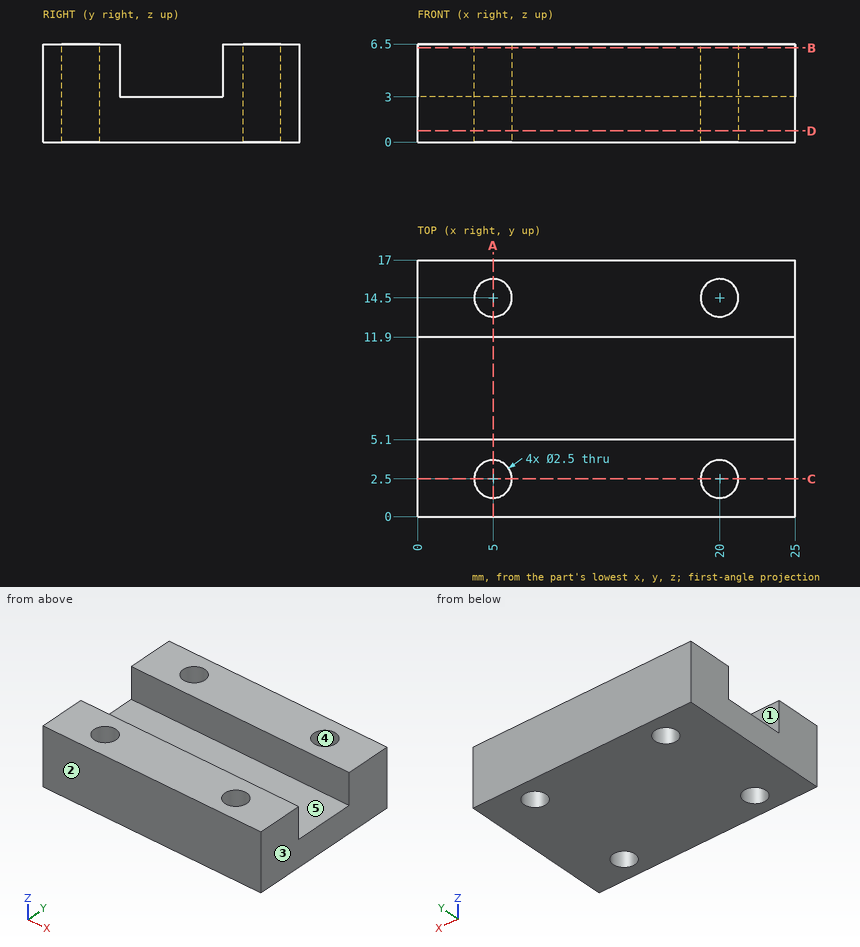
Print and shaded views of the part. All mm, measured from the part's lowest x, y and z. A direction names the side the tool comes from. Give positions to 0.01 mm unless a question says otherwise; leave off trailing zeros. Order: outer loops, then holes, each group sorted by start corner. A loop starts at its lowest first (then second) coordinate and runs counter-clockwise, first axis right, second up. Notation, with made-up numbers: (23, 86.5) - (76, 86.5) arc R22 ccw to (76, 101.5) - close; hole circle Ø4 at (14, 27.5). An arc over 180 degrees is marked (long way). Use a Markdown table: item, result.
1) Saw through at D-D on z = 0.75. List the corners of the cut face in (x, y).
Checked values:
| item | result |
|---|---|
| outline | (0, 0) - (25, 0) - (25, 17) - (0, 17) - close; hole circle Ø2.5 at (5, 2.5); hole circle Ø2.5 at (5, 14.5); hole circle Ø2.5 at (20, 2.5); hole circle Ø2.5 at (20, 14.5) |
2) Saw through at B-B on z = 6.25. List the corners of the cut face in (x, y).
Checked values:
| item | result |
|---|---|
| outline | (0, 0) - (25, 0) - (25, 5.1) - (0, 5.1) - close; (0, 11.9) - (25, 11.9) - (25, 17) - (0, 17) - close; hole circle Ø2.5 at (5, 2.5); hole circle Ø2.5 at (5, 14.5); hole circle Ø2.5 at (20, 2.5); hole circle Ø2.5 at (20, 14.5) |
3) 3-axis set-ups, long thin cutter, end or side, ignore diameter. For the marked faces 4 and 5: which of +Z, -Z, +X, -X, +Y, -Y reach the whole face in a straight line?
Checked values:
| item | result |
|---|---|
| face 4 | +Z, -Z |
| face 5 | +Z, +X, -X |
4) Two-plate mould, pull along Y, no slides. Class the marked faces 1, 2 and 3: +Y half, -Y half, draft (parallel to the pull), parting line (faces both ways), or undercut.
Checked values:
| item | result |
|---|---|
| face 1 | undercut |
| face 2 | -Y half |
| face 3 | draft |
5) Saw through at C-C on y = 2.5. List the corners of the cut face in (x, z).
Checked values:
| item | result |
|---|---|
| outline | (0, 0) - (3.75, 0) - (3.75, 6.5) - (0, 6.5) - close; (6.25, 0) - (18.75, 0) - (18.75, 6.5) - (6.25, 6.5) - close; (21.25, 0) - (25, 0) - (25, 6.5) - (21.25, 6.5) - close |
6) Saw through at A-A on x = 5. List the corners of the cut face in (y, z).
Checked values:
| item | result |
|---|---|
| outline | (0, 0) - (1.25, 0) - (1.25, 6.5) - (0, 6.5) - close; (3.75, 0) - (13.25, 0) - (13.25, 6.5) - (11.9, 6.5) - (11.9, 3) - (5.1, 3) - (5.1, 6.5) - (3.75, 6.5) - close; (15.75, 0) - (17, 0) - (17, 6.5) - (15.75, 6.5) - close |
7) Flat gauge pin, fed straight in: P1, Ø2, axis at y = 10.5, z = 4.5, coming from the -X side. Where does the tip first touch, or does it go through?
Checked values:
| item | result |
|---|---|
| P1 | through |
8) Probe L1, parallel to Y at x = 5, z = 3.5; L2, parallel to Y at x = 5, z = 2.25; L3, parallel to Y at x = 16.5, z = 4.75. List the from-to ranges inside material, lowest first. Write a range as from..to.
Checked values:
| item | result |
|---|---|
| L1 | 0..1.25, 3.75..5.1, 11.9..13.25, 15.75..17 |
| L2 | 0..1.25, 3.75..13.25, 15.75..17 |
| L3 | 0..5.1, 11.9..17 |
